from build123d import *

# Parameters (mm, degrees)
BASE_PLATE_DEPTH              = 85
PIVOT_BOSS_SKETCH_R           = 20
PIVOT_BOSS_DEPTH              = 30
GUSSET_RIB_DEPTH              = 10
BOSS_SUPPORT_BLOCK_REACH      = 113.557
BOSS_SUPPORT_BLOCK_END_RADIUS = 20
BOSS_SUPPORT_BLOCK_SKETCH_W   = 15
BOSS_SUPPORT_BLOCK_SKETCH_H   = 10
PIVOT_BORE_SKETCH_R           = 10
PIVOT_BORE_20_DEPTH           = 115.127122105
MOUNTING_HOLES_SKETCH_R       = 5.697054252
MOUNTING_HOLES_SKETCH_R_2     = 5.829543886
MOUNTING_HOLES_2X_DEPTH       = 112.557160236
CORNER_FILLETS_R5_R           = 5


with BuildPart() as part:
    # Base Plate Profile Sketch → Base Plate (new body)
    with BuildSketch(Plane.XY):
        Polygon((0, 0), (0, 16), (48, 16), (48, 4), (8, 4), (8, 0), align=None)
    extrude(amount=BASE_PLATE_DEPTH)



with BuildPart() as body_2:
    # Pivot Boss Sketch → Pivot Boss (new body)
    with BuildSketch(Plane.ZY):
        with Locations(Location((42.5, 50, 0), (0, 0, 270))):
            Circle(PIVOT_BOSS_SKETCH_R)
    extrude(amount=-PIVOT_BOSS_DEPTH)


with BuildPart() as part_1:
    add(part.part)

    add(body_2.part)  # Gusset Rib merges body 2
    # Gusset Rib Sketch → Gusset Rib (add)
    with BuildSketch(Plane.ZY):
        with BuildLine():
            Line((24.625908668, 58.973118691), (0, 16))
            Line((0, 16), (85, 16))
            Line((85, 16), (60.374091332, 58.973118691))
            ThreePointArc((60.374091332, 58.973118691), (61.961267002, 54.610757712), (62.5, 50))
            ThreePointArc((62.5, 50), (37.889242288, 30.538732998), (24.625908668, 58.973118691))
        make_face()
    extrude(amount=-GUSSET_RIB_DEPTH)

    # Boss Support Block: up to this cylinder (the profile starts outside it)
    boss_support_block_end = Plane(origin=(17.5, 50, 42.5), z_dir=(-1, 0, 0)) * Cylinder(BOSS_SUPPORT_BLOCK_END_RADIUS, 268.114, mode=Mode.PRIVATE)
    # Boss Support Block Sketch → Boss Support Block (add, up to the surface)
    with BuildSketch(Plane(origin=(0, 16, 0), x_dir=(1, 0, 0), z_dir=(0, 1, 0)), mode=Mode.PRIVATE) as boss_support_block_sk1:
        with Locations((17.5, -42.5)):
            Rectangle(BOSS_SUPPORT_BLOCK_SKETCH_W, BOSS_SUPPORT_BLOCK_SKETCH_H)
    boss_support_block_tool1 = extrude(boss_support_block_sk1.sketch, amount=BOSS_SUPPORT_BLOCK_REACH, mode=Mode.PRIVATE) - boss_support_block_end
    add(boss_support_block_tool1.solids().sort_by_distance((17.5, 16, 42.5))[0])

    # Pivot Bore Sketch → Pivot Bore Ø20 (cut, through all)
    with BuildSketch(Plane(origin=(30, 0, 0), x_dir=(0, 0, -1), z_dir=(1, 0, 0))):
        with Locations(Location((-42.5, 50, 0), (0, 0, 90))):
            Circle(PIVOT_BORE_SKETCH_R)
    extrude(amount=-PIVOT_BORE_20_DEPTH, mode=Mode.SUBTRACT)

    # Mounting Holes Sketch → Mounting Holes 2x (cut, through all)
    with BuildSketch(Plane(origin=(0, 16, 0), x_dir=(1, 0, 0), z_dir=(0, 1, 0))):
        with Locations(Location((30, -12.5, 0), (0, 0, 180))):
            Circle(MOUNTING_HOLES_SKETCH_R)
        with Locations(Location((30, -72.5, 0), (0, 0, 180))):
            Circle(MOUNTING_HOLES_SKETCH_R_2)
    extrude(amount=-MOUNTING_HOLES_2X_DEPTH, mode=Mode.SUBTRACT)

    # Corner Fillets R5
    corner_fillets_r5_edges = [part_1.edges().sort_by_distance(p)[0] for p in [
        (48, 10, 85),
        (48, 10, 0),
    ]]
    fillet(corner_fillets_r5_edges, radius=CORNER_FILLETS_R5_R)


solid = part_1.part
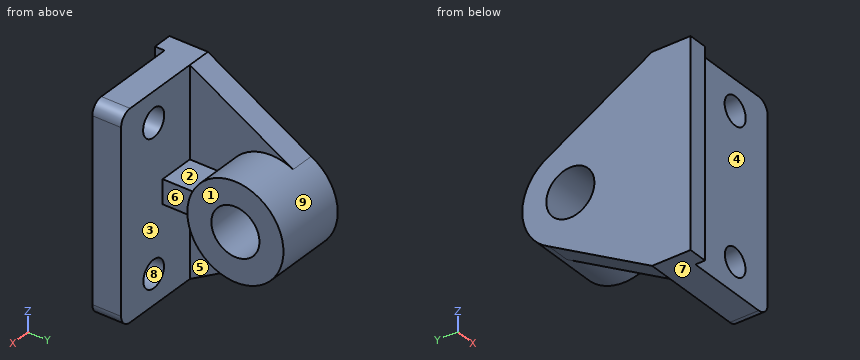
Input: part model. Units: mm. Frame: model coordinates. Face numbers are marked on the shaded views. A direction names the side the tool comes from. Coordinates: 2 decimals unless noted, no trailing zeros. Order: outer loops, then holes, each group sorted by start corner. A loop starts at its lowest first (then second) coordinate and runs counter-clockwise, first axis right, second up. Notation, with made-up numbers: M -24.75,-26 L 27.25,-26 A20 ccw 27.25,7 Z; hole C 57,30 d2. An arc over 180 degrees is marked long. Answer in a Markdown table with one row per item.
(1) Material intervals for line 1 (Z direction, x = 30, y = 7); line 2 (Z direction, x = 34.5, y = 8.5); line 3 (Z direction, x = 19, y = 50), sorted ascending. Write a range as [from, to].
Numbers:
| item | result |
|---|---|
| line 1 | z = [0, 6.8], [18.2, 66.67], [78.33, 85] |
| line 2 | z = [0, 9.01], [15.99, 68.79], [76.21, 85] |
| line 3 | z = [22.5, 32.5], [52.5, 62.5] |
(2) Section query C-C, the plane y = 54. Output: boundary loops of the cut face in (x, z), plus the area to 3 significant figures.
Numbers:
| item | result |
|---|---|
| outline | M 0,21.78 L 10,21.78 L 10,22.9 L 30,22.9 L 30,33.33 L 0,33.33 Z; M 0,51.67 L 30,51.67 L 30,62.1 L 10,62.1 L 10,63.22 L 0,63.22 Z |
| area | 648 mm^2 |
(3) Section query A-A, the plane x = 22. Output: boundary loops of the cut face in (y, z), plus the area to 3 significant figures.
Numbers:
| item | result |
|---|---|
| outline | M 4,0 L 16,0 L 16,37.5 L 30.64,37.5 A20 ccw long 30.64,47.5 L 16,47.5 L 16,85 L 4,85 Z; hole C 50,42.5 d20 |
| area | 2,100 mm^2 |
(4) Section query B-B, the plane z = 42.5. Output: boundary loops of the cut face in (x, y).
Numbers:
| item | result |
|---|---|
| outline | M 0,0 L 8,0 L 8,4 L 48,4 L 48,16 L 25,16 L 25,30 L 30,30 L 30,40 L 0,40 Z; M 0,60 L 30,60 L 30,70 L 0,70 Z |
(5) Draft query along Z for the marked faces 6, 7, 8 and 9. Return one class per face: pulls with the +Z half, pulls with the -Z half, needs draft (parallel to the pull), parting line crosses it, or undercut.
Numbers:
| item | result |
|---|---|
| face 6 | needs draft |
| face 7 | pulls with the -Z half |
| face 8 | undercut |
| face 9 | parting line crosses it |
(6) Section query D-D, the plane x = 28. Output: boundary loops of the cut face in (y, z).
Numbers:
| item | result |
|---|---|
| outline | M 4,0 L 16,0 L 16,7.17 L 4,7.17 Z; M 4,17.83 L 16,17.83 L 16,67.02 L 4,67.02 Z; M 4,77.98 L 16,77.98 L 16,85 L 4,85 Z; C 50,42.5 d40; hole C 50,42.5 d20 |
(7) Access query for the marked faces 1, 2, 3, 4 and 5. Directions: +Z, -Z, +X, -X, +Y, -Y. A direction counts if a zero-diameter tool reaches every point of the face in a straight line with its end or side. Return the directions, or none.
Numbers:
| item | result |
|---|---|
| face 1 | +Z, -Z, +X, +Y |
| face 2 | +Z, +X |
| face 3 | +X |
| face 4 | +Z, -Z, +X, -Y |
| face 5 | -Z, +X |
(8) Contact query for flat-ended pins moving along their axis: pin 1 Ø3 at (y, z) = (44, 26) entering from -X; pin 2 Ø1.5 at (x, y) = (12, 55) entering from -Z; pin 3 Ø3 at (x, z) = (26, 27) entering from -Y; pin 4 Ø1 at (x, z) = (38.5, 66) entering from +Y. Output: stop coordinate, or through.
Numbers:
| item | result |
|---|---|
| pin 1 | stops at x = 0 |
| pin 2 | stops at z = 22.96 |
| pin 3 | stops at y = 4 |
| pin 4 | stops at y = 16 |
